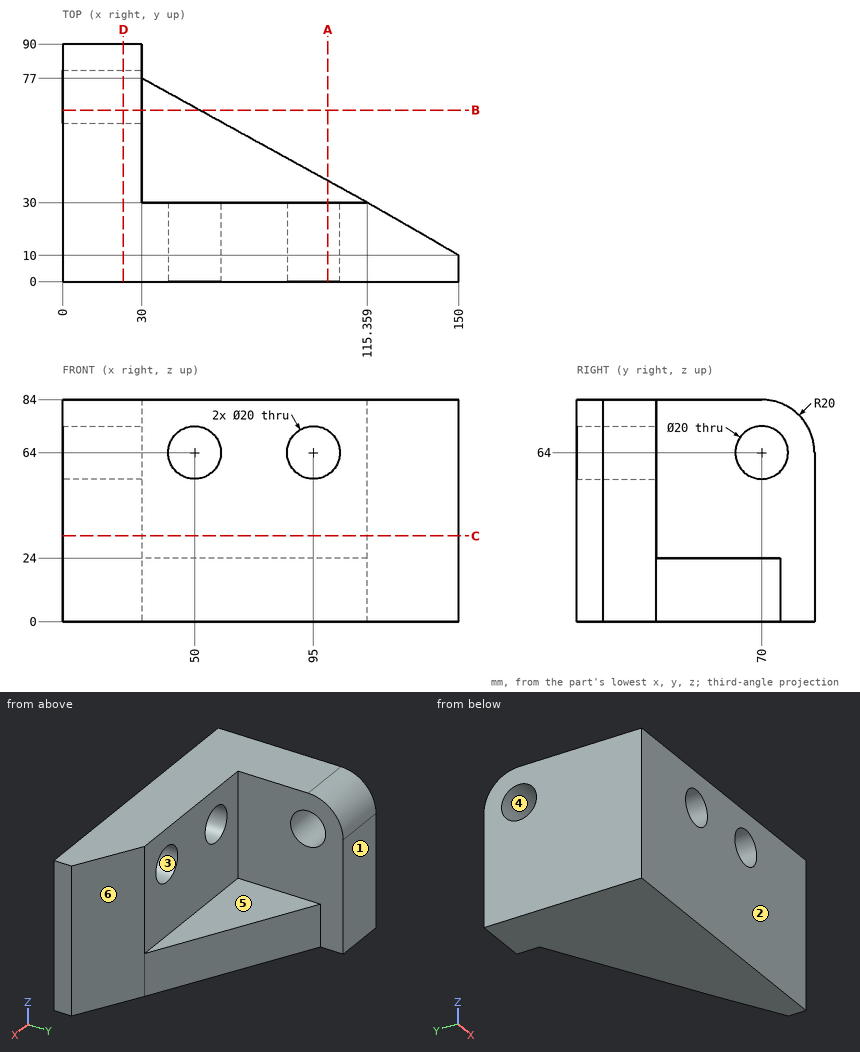
Check sheet for the drawn part. Datum: minimum x, y, z corner. Units: mm. A direction names the side the tool comes from. Round coordinates to 2 decimals unless told otherwise and drop trailing zeros. Order: outer loops, then holes, each group sorted by start corner. A loop starts at its lowest first (then second) coordinate and runs counter-clockwise, first axis right, second up.
(1) Scan lines: probe 1 along Z at (x, y) = (50, 12); probe 2 along Y at (x, z) = (17, 64); probe 3 along Y at (x, z) = (72.5, 67). Record each from-to range of solid material in increasing order.
(2) Access from +Z, -Z, +X, -X, +Y, -Y to the whole of each face (thin tool, end or side, straight path). Record for the marked faces 5 and 6.
(3) Cross-section at B-B, the plane y = 65. Enter the section's corners in (x, z), and give its area (3 significant figures).
(4) Draft check along Y on the marked faces 1, 2, 3 and 4. Enter one of: pulls with the +Y half, pulls with the -Y half, needs draft (parallel to the pull), parting line crosses it, or undercut.
(5) Cross-section at A-A, the plane x = 100.5. Enter the section's corners in (y, z), and give its area (3 significant figures).
(6) Cross-section at D-D, the plane x = 23. Enter the section's corners in (y, z).
(7) Go/stop test with flat-tipped pins: P1, Ø12, axis at x = 95, z = 64, coming from the +Y side; P2, Ø12, axis at x = 124.5, z = 62, coming from the +Y side; P3, Ø8, axis at y = 14.5, z = 9, coming from the -X side; P4, Ø5, axis at y = 19.5, z = 40, coming from the +X side. Record where each tip stops, or that it passes through.
(8) Cross-section at C-C, the plane z = 32.5. Enter the section's corners in (x, y).
Check sheet entries:
1. probe 1: z = 0 to 54, 74 to 84
1. probe 2: y = 0 to 60, 80 to 90
1. probe 3: y = 0 to 30
2. face 5: +Z, +X, +Y
2. face 6: +Z, -Z, +X, +Y
3. outline: (0, 0) - (51.79, 0) - (51.79, 24) - (30, 24) - (30, 55.34) - (0, 55.34) - close; (0, 72.66) - (30, 72.66) - (30, 84) - (0, 84) - close
3. area: 2,520 mm2
4. face 1: pulls with the +Y half
4. face 2: pulls with the -Y half
4. face 3: needs draft
4. face 4: undercut
5. outline: (0, 0) - (38.18, 0) - (38.18, 24) - (30, 24) - (30, 55.65) - (0, 55.65) - close; (0, 72.35) - (30, 72.35) - (30, 84) - (0, 84) - close
5. area: 2,220 mm2
6. outline: (0, 0) - (90, 0) - (90, 64) arc R20 ccw to (70, 84) - (0, 84) - close; hole circle Ø20 at (70, 64)
7. P1: passes through
7. P2: stops at y = 28.19
7. P3: stops at x = 0
7. P4: stops at x = 137.88
8. outline: (0, 0) - (150, 0) - (150, 10) - (115.36, 30) - (30, 30) - (30, 90) - (0, 90) - close
